from build123d import *

# Parameters (mm, degrees)
SKETCH1_R               = 5
BOSS_EXTRUDE1_DEPTH     = 75
CUT_EXTRUDE1_DEPTH      = 76.332595867
CUT_EXTRUDE1_DEPTH_BACK = 76.332595867
SKETCH2_W               = 68
SKETCH2_H               = 14.535467824
CUT_EXTRUDE2_START      = -12
SKETCH3_R               = 5
SKETCH3_R_2             = 3.125
CUT_EXTRUDE2_DEPTH      = 12
SKETCH4_OUTSIDE_W       = 42.134
SKETCH4_OUTSIDE_H       = 42.134
CUT_EXTRUDE3_DEPTH      = 12
SKETCH5_OUTSIDE_W       = 42.134
SKETCH5_OUTSIDE_H       = 42.134
SKETCH5_OUTSIDE_R       = 4
CUT_EXTRUDE4_DEPTH      = 10
SKETCH6_W               = 10.564036003
SKETCH6_H               = 1.244008039
CUT_EXTRUDE5_DEPTH      = 5
SKETCH31_W              = 1.1
SKETCH31_H              = 0.2
SKETCH32_W              = 1.1
SKETCH32_H              = 0.2


with BuildPart() as part:
    # Sketch1 → Boss-Extrude1 (new, symmetric)
    with BuildSketch(Plane.XY):
        Circle(SKETCH1_R)
    extrude(amount=BOSS_EXTRUDE1_DEPTH, both=True)

    # Sketch2 → Cut-Extrude1 (cut, two sides: drawn at the far end of the back side and taken through both)
    with BuildSketch(Plane(origin=(0, 0, 0), x_dir=(0, 0, -1), z_dir=(1, 0, 0)).offset(-CUT_EXTRUDE1_DEPTH_BACK)):
        with Locations((0, 10.467733912)):
            Rectangle(SKETCH2_W, SKETCH2_H)
    extrude(amount=CUT_EXTRUDE1_DEPTH + CUT_EXTRUDE1_DEPTH_BACK, mode=Mode.SUBTRACT)

    # Sketch3 → Cut-Extrude2 (cut)
    with BuildSketch(Plane(origin=(0, 0, -75), x_dir=(-1, 0, 0), z_dir=(0, 0, -1)).offset(CUT_EXTRUDE2_START)):
        Circle(SKETCH3_R)
        Circle(SKETCH3_R_2, mode=Mode.SUBTRACT)
    extrude(amount=CUT_EXTRUDE2_DEPTH, mode=Mode.SUBTRACT)

    # Sketch4 outside → Cut-Extrude3 (cut)
    with BuildSketch(Plane(origin=(0, 0, -75), x_dir=(-1, 0, 0), z_dir=(0, 0, -1))):
        Rectangle(SKETCH4_OUTSIDE_W, SKETCH4_OUTSIDE_H)
        with BuildLine():
            Line((-1.957198253, 2.5), (1.957198253, 2.5))
            ThreePointArc((1.957198253, 2.5), (0, -3.175), (-1.957198253, 2.5))
        make_face(mode=Mode.SUBTRACT)
    extrude(amount=-CUT_EXTRUDE3_DEPTH, mode=Mode.SUBTRACT)

    # Sketch5 outside → Cut-Extrude4 (cut)
    with BuildSketch(Plane.XY.offset(75)):
        Rectangle(SKETCH5_OUTSIDE_W, SKETCH5_OUTSIDE_H)
        Circle(SKETCH5_OUTSIDE_R, mode=Mode.SUBTRACT)
    extrude(amount=-CUT_EXTRUDE4_DEPTH, mode=Mode.SUBTRACT)

    # Sketch6 → Cut-Extrude5 (cut)
    with BuildSketch(Plane.XY.offset(75)):
        with Locations((0.265856556, 3.982832188)):
            Rectangle(SKETCH6_W, SKETCH6_H)
    extrude(amount=-CUT_EXTRUDE5_DEPTH, mode=Mode.SUBTRACT)

    # Sketch31 → Cut-Revolve1 (revolve, cut)
    with BuildSketch(Plane(origin=(-100, 0, -63), x_dir=(0, 0, 1), z_dir=(0, 1, 0))):
        with Locations((11.45, 95.1)):
            Rectangle(SKETCH31_W, SKETCH31_H)
    revolve(axis=Axis((0, 0, -63), (0, 0, 1)), mode=Mode.SUBTRACT)

    # Sketch32 → Cut-Revolve11 (revolve, cut)
    with BuildSketch(Plane(origin=(100, 0, 65), x_dir=(0, 0, -1), z_dir=(0, 1, 0)), mode=Mode.PRIVATE) as cut_revolve11_sk:
        with Locations((7.45, 95.1)):
            Rectangle(SKETCH32_W, SKETCH32_H)
    revolve(cut_revolve11_sk.sketch.rotate(Axis((0, 0, 65), (0, 0, -1)), 180), axis=Axis((0, 0, 65), (0, 0, -1)), mode=Mode.SUBTRACT)


solid = part.part
Geometry: final body of the model. Coordinates: model frame, mm. A direction names the side the tool comes from. Coordinates: 2 decimals unless noted, no trailing zeros. Order: outer loops, then holes, each group sorted by start corner. A loop starts at its lowest first (then second) coordinate and runs counter-clockwise, first axis right, second up.
1) Draft query along Z for faces 1 (the flat face through (0, 0, -75)), 2 (the flat face through (0, 3.2, 0)), 3 (the cylindrical face through (-4.58, -1.44, -51.54)), 4 (the flat face through (0, 2.5, -69)). Return one class per face: released by +Z, released by -Z, zero draft, split by the parting line, or undercut.
Result sheet:
face 1: released by -Z
face 2: undercut
face 3: undercut
face 4: zero draft
2) First-contact query: P1, Ø3.5, axis at x = 0, z = 72.5, coming from the +Y side; P2, Ø1.9, axis at x = 1, z = -67, coming from the +Y side; P3, Ø2.5, axis at x = 0.5, z = 6, coming from the +Y side. Flat tips, straight axial feed; report the tip coordinate or a pass-through.
Result sheet:
P1: stops at y = 3.36
P2: stops at y = 2.5
P3: stops at y = 3.2
3) Section B-B (y = 0). Return loops of the section in (x, z) (3 decimals).
Result sheet:
outline: (-5, -63) - (-3.125, -63) - (-3.125, -75) - (3.125, -75) - (3.125, -63) - (5, -63) - (5, -52.1) - (4.8, -52.1) - (4.8, -51) - (5, -51) - (5, 57) - (4.8, 57) - (4.8, 58.1) - (5, 58.1) - (5, 65) - (4, 65) - (4, 75) - (-4, 75) - (-4, 65) - (-5, 65) - (-5, 58.1) - (-4.8, 58.1) - (-4.8, 57) - (-5, 57) - (-5, -51) - (-4.8, -51) - (-4.8, -52.1) - (-5, -52.1) - close
4) Ray query, probe 1 along Z at (x, y) = (3.25, -3.75); probe 2 along Z at (x, y) = (3.5, -2); probe 3 along X at (y, z) = (-1, 66). Return the intervals inside material, ascending.
Result sheet:
probe 1: z = -63 to -52.1, -51 to 57, 58.1 to 65
probe 2: z = -63 to 65
probe 3: x = -3.87 to 3.87
5) Section D-D (z = 2). Return loops of the section in (x, y), then the cut area to 3 significant figures.
Result sheet:
outline: (-3.84, 3.2) arc R5 ccw (long way) to (3.84, 3.2) - close
area: 68.9 mm2
6) Set-up query: faces 5 (the cylindrical face through (-4.58, 1.44, 57.54)), 6 (the cylindrical face through (0.109, -3.123, -68.916)), 7 (the flat face through (0, 3.361, 73)). Return all of +Z, -Z, +X, -X, +Y, -Y with unobstructed straight access to the full face (end or side cutting, diameter ignored); none if empty.
Result sheet:
face 5: none
face 6: -Z
face 7: +Z, +X, -X, +Y
7) Section C-C (z = -45.5). Return loops of the section in (x, y).
Result sheet:
outline: circle Ø10 at (0, 0)
